Input: dimensioned drawing with shaded views. Units: mm. Origin: part minimum x, y, z. A direction names the side the tool comes from. Coordinates: 2 decimals unless noted, no trailing zeros. Order: outer loops, then holes, each group sorted by start corner. A loop starts at its lowest first (then second) coordinate and runs counter-clockwise, first axis right, second up. Notation, with made-up numbers: (16, -2.5) -> (43, -2.5) arc R29 ccw to (43, 21.5) -> close; hole circle Ø1 at (-34, -8.5). An arc over 180 degrees is marked (long way). Answer as CSV lines item,"result".
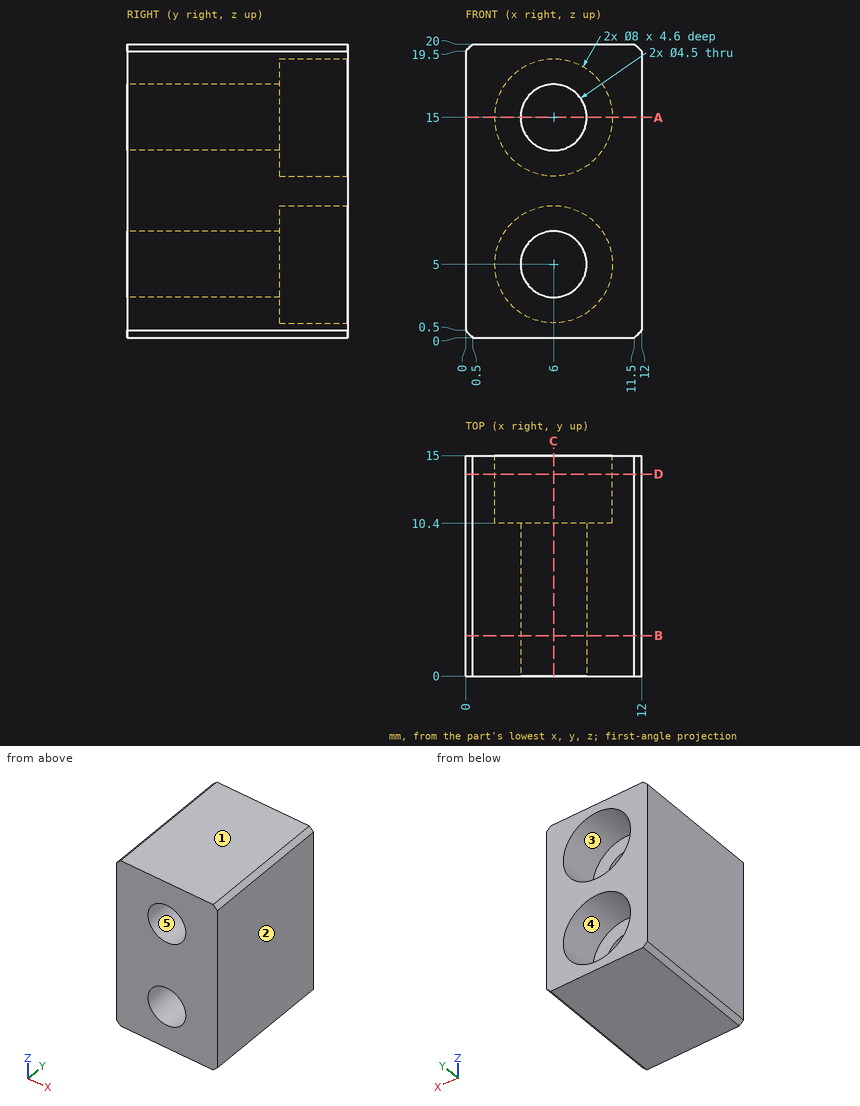
1. Cut plane A-A (z = 15). Return the cut outline in (x, y), plus the area to 3 significant figures.
Findings:
outline,"(0, 0) -> (3.75, 0) -> (3.75, 10.4) -> (2, 10.4) -> (2, 15) -> (0, 15) -> close; (8.25, 0) -> (12, 0) -> (12, 15) -> (10, 15) -> (10, 10.4) -> (8.25, 10.4) -> close"
area,"96.4 mm2"
2. Cut plane C-C (x = 6). Return the cut outline in (y, z).
Findings:
outline,"(0, 0) -> (15, 0) -> (15, 1) -> (10.4, 1) -> (10.4, 2.75) -> (0, 2.75) -> close; (0, 7.25) -> (10.4, 7.25) -> (10.4, 9) -> (15, 9) -> (15, 11) -> (10.4, 11) -> (10.4, 12.75) -> (0, 12.75) -> close; (0, 17.25) -> (10.4, 17.25) -> (10.4, 19) -> (15, 19) -> (15, 20) -> (0, 20) -> close"
3. Ray query, line 1 along Z through (x, y) = (6, 13.95); line 2 along Z through (x, y) = (6, 7.5); line 3 along X through (y, z) = (12.65, 15). Return the intervals inside material, ascending.
Findings:
line 1,"z = 0 to 1, 9 to 11, 19 to 20"
line 2,"z = 0 to 2.75, 7.25 to 12.75, 17.25 to 20"
line 3,"x = 0 to 2, 10 to 12"
4. Reachability of the marked faces 4 and 5 from +Z, -Z, +X, -X, +Y, -Y: full face, straight path, thin tool, end or side. Return the list, or none.
Findings:
face 4,"+Y"
face 5,"+Y, -Y"
5. Contact query for a flat-ended pin moving along its axis: pin 1 (6.5 mm diameter, centred on x = 6, z = 5, fed in from +Y). Output: stop coordinate, or through.
Findings:
pin 1,"stops at y = 10.4"
6. Mould query, pull axis X, two halves, no side actions, for the marked faces 1, 2 and 3. Classes: released by +X, released by -X, zero draft, split by the parting line, or undercut.
Findings:
face 1,"zero draft"
face 2,"released by +X"
face 3,"undercut"
7. Cut plane D-D (y = 13.75). Return the cut outline in (x, z).
Findings:
outline,"(0, 0.5) -> (0.5, 0) -> (11.5, 0) -> (12, 0.5) -> (12, 19.5) -> (11.5, 20) -> (0.5, 20) -> (0, 19.5) -> close; hole circle Ø8 at (6, 5); hole circle Ø8 at (6, 15)"
8. Cut plane B-B (y = 2.75). Return the cut outline in (x, z).
Findings:
outline,"(0, 0.5) -> (0.5, 0) -> (11.5, 0) -> (12, 0.5) -> (12, 19.5) -> (11.5, 20) -> (0.5, 20) -> (0, 19.5) -> close; hole circle Ø4.5 at (6, 5); hole circle Ø4.5 at (6, 15)"
